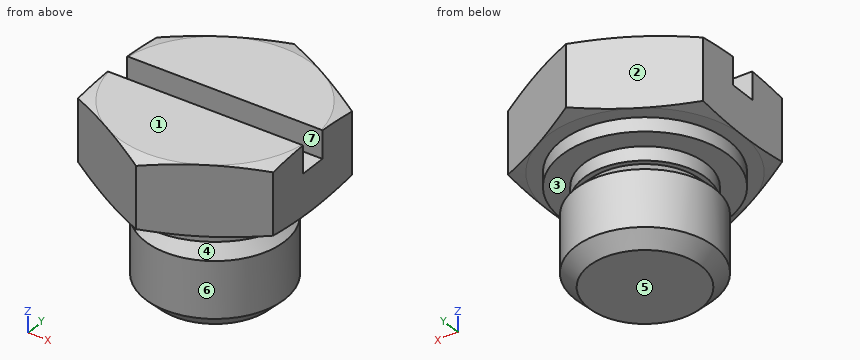
from build123d import *

# Parameters (mm, degrees)
SKETCH_2_R          = 5
CUT_EXTRUDE_1_DEPTH = 3
SKETCH_3_W          = 10
SKETCH_3_H          = 1
CUT_EXTRUDE_2_DEPTH = 1


with BuildPart() as part:
    # 草图1 → 旋转1 (revolve)
    with BuildSketch(Plane(origin=(0, 0, 0), x_dir=(0, 0, -1), z_dir=(1, 0, 0)), mode=Mode.PRIVATE) as revolve_1_sk:
        Polygon((-3, 0), (-3, 3.5), (-2.598076211, 5), (-0.901923789, 5), (-0.5, 3.5), (-0.5, 3), (0, 3), (0, 2.2), (0.5, 2.2), (0.5, 2.0095), (0.9905, 2.5), (3.0095, 2.5), (3.5, 2.0095), (3.5, 0), align=None)
    revolve(revolve_1_sk.sketch.rotate(Axis((0, 0, -3.5), (0, 0, 1)), 270), axis=Axis((0, 0, -3.5), (0, 0, 1)))

    # 草图2 → 切除-拉伸1 (cut)
    with BuildSketch(Plane.XY):
        Circle(SKETCH_2_R)
        Polygon((-3.5, 2.020725942), (-3.5, -2.020725942), (0, -4.041451884), (3.5, -2.020725942), (3.5, 2.020725942), (0, 4.041451884), align=None, mode=Mode.SUBTRACT)
    extrude(amount=CUT_EXTRUDE_1_DEPTH, mode=Mode.SUBTRACT)

    # 草图3 → 切除-拉伸2 (cut)
    with BuildSketch(Plane.XY.offset(3)):
        Rectangle(SKETCH_3_W, SKETCH_3_H)
    extrude(amount=-CUT_EXTRUDE_2_DEPTH, mode=Mode.SUBTRACT)


solid = part.part
Can you work these out from the model? Positions are in its coordinate system, mm. Face numbers are marked on the shaded views. A direction names the side the tool comes from. Round coordinates to 2 decimals unless told otherwise and drop trailing zeros. Write each loop counter-clockwise with the first axis right and the second up, starting at its lowest first coordinate (ties: lowest second). Pieces come first, ordered by that corner, then holes. Notation, with made-up numbers: M 65.25,-29.5 L 76.25,-29.5 A17 cw 76.25,-1.5 Z; hole C -22.75,71 d4. An arc over 180 degrees is marked long. Use a Markdown table: item, result.
Item 1: If I drill on line 1 along Z through (x, y) = (-1.5, 0.25); line 2 along Y through (x, z) = (0, -2.5); line 3 along Z through (x, y) = (-0.5, 2.75), over which ranges is the centre line in solid material (lowest first)? Write a range as [from, to].
Found:
| item | result |
|---|---|
| line 1 | z = [-3.5, 2] |
| line 2 | y = [-2.5, 2.5] |
| line 3 | z = [0, 3] |
Item 2: For pin 1 Ø1.5 at (x, z) = (1, 0.5) entering from -Y; pin 2 Ø3 at (y, z) = (0.5, -2.5) entering from -X; pin 3 Ø0.8 at (x, y) = (0.5, 0) entering from +Z, each with a flat end and sliding along its axis, tell me the tip position at first contact or that it passes through.
Found:
| item | result |
|---|---|
| pin 1 | stops at y = -3.89 |
| pin 2 | stops at x = -2.5 |
| pin 3 | stops at z = 2 |
Item 3: Which directions (+Z, -Z, +X, -X, +Y, -Y) give clear straight access to the entire face, cutting with the end or side of a thin tool? Please do the marked faces 4, 5, 6 and 7.
Found:
| item | result |
|---|---|
| face 4 | none |
| face 5 | -Z, +X, -X, +Y, -Y |
| face 6 | -Z |
| face 7 | +Z, +X, -X |
Item 4: I want a section at B-B (z = 1.25). List the corners of the cut face in (x, y) for me, and give its area (3 significant figures).
Found:
| item | result |
|---|---|
| outline | M -3.5,-2.02 L 0,-4.04 L 3.5,-2.02 L 3.5,2.02 L 0,4.04 L -3.5,2.02 Z |
| area | 42.4 mm2 |
Item 5: I want a section at C-C (z = -2). List the corners of the cut face in (x, y) for me, and give its area (3 significant figures).
Found:
| item | result |
|---|---|
| outline | C 0,0 d5 |
| area | 19.6 mm2 |
Item 6: I want a section at D-D (z = -0.75). List the corners of the cut face in (x, y) for me.
Found:
| item | result |
|---|---|
| outline | C 0,0 d4.52 |
Item 7: We'd pull the mould along Z, two halves only. Please class the marked faces 1, 2 and 3: released by +Z, released by -Z, zero draft, split by the parting line, or undercut.
Found:
| item | result |
|---|---|
| face 1 | released by +Z |
| face 2 | zero draft |
| face 3 | undercut |
Item 8: I want a section at A-A (z = 2.5). List the corners of the cut face in (x, y) for me, and give its area (3 significant figures).
Found:
| item | result |
|---|---|
| outline | M -3.5,-2.02 L 0,-4.04 L 3.5,-2.02 L 3.5,-0.5 L -3.5,-0.5 Z; M -3.5,0.5 L 3.5,0.5 L 3.5,2.02 L 0,4.04 L -3.5,2.02 Z |
| area | 35.4 mm2 |
